from build123d import *

# Parameters (mm, degrees)
BASE_PLATE_SKETCH_W        = 120
BASE_PLATE_SKETCH_H        = 50
BASE_PLATE_120X50X10_DEPTH = 10
CLAMP_BOSS_DEPTH           = 22
BORE_SKETCH_R              = 10
BORE_20_DEPTH              = 22
COUNTERBORE_SKETCH_R       = 6
COUNTERBORES_2X_12_DEPTH   = 5
BOLT_HOLE_SKETCH_R         = 3
BOLT_HOLES_2X_6_DEPTH      = 25
MOUNTING_HOLE_SKETCH_R     = 5
MOUNTING_HOLES_4X_10_DEPTH = 25
CORNER_CHAMFERS_5MM_SIZE   = 5


with BuildPart() as part:
    # Base Plate Sketch → Base Plate 120x50x10 (new body)
    with BuildSketch(Plane.XY):
        Rectangle(BASE_PLATE_SKETCH_W, BASE_PLATE_SKETCH_H)
    extrude(amount=BASE_PLATE_120X50X10_DEPTH)

    # Clamp Boss Sketch → Clamp Boss (add)
    with BuildSketch(Plane.XY.offset(10)):
        Polygon((20, 8.3), (35, 8.3), (35, -8.3), (20, -8.3), (8.3, -20), (-8.3, -20), (-20, -8.3), (-35, -8.3), (-35, 8.3), (-20, 8.3), (-8.3, 20), (8.3, 20), align=None)
    extrude(amount=CLAMP_BOSS_DEPTH)

    # Bore Sketch → Bore Ø20 (cut)
    with BuildSketch(Plane.XY.offset(32)):
        Circle(BORE_SKETCH_R)
    extrude(amount=-BORE_20_DEPTH, mode=Mode.SUBTRACT)

    # Counterbore Sketch → Counterbores 2xØ12 (cut)
    with BuildSketch(Plane.XY.offset(32)):
        with Locations((-26, 0)):
            Circle(COUNTERBORE_SKETCH_R)
        with Locations((26, 0)):
            Circle(COUNTERBORE_SKETCH_R)
    extrude(amount=-COUNTERBORES_2X_12_DEPTH, mode=Mode.SUBTRACT)

    # Bolt Hole Sketch → Bolt Holes 2xØ6 (cut)
    with BuildSketch(Plane.XY.offset(27)):
        with Locations((-26, 0)):
            Circle(BOLT_HOLE_SKETCH_R)
        with Locations((26, 0)):
            Circle(BOLT_HOLE_SKETCH_R)
    extrude(amount=-BOLT_HOLES_2X_6_DEPTH, mode=Mode.SUBTRACT)

    # Mounting Hole Sketch → Mounting Holes 4xØ10 (cut)
    with BuildSketch(Plane.XY.offset(10)):
        with Locations((50, 15)):
            Circle(MOUNTING_HOLE_SKETCH_R)
        with Locations((50, -15)):
            Circle(MOUNTING_HOLE_SKETCH_R)
        with Locations((-50, 15)):
            Circle(MOUNTING_HOLE_SKETCH_R)
        with Locations((-50, -15)):
            Circle(MOUNTING_HOLE_SKETCH_R)
    extrude(amount=-MOUNTING_HOLES_4X_10_DEPTH, mode=Mode.SUBTRACT)

    # Corner Chamfers 5mm
    corner_chamfers_5mm_edges = [part.edges().sort_by_distance(p)[0] for p in [
        (60, -25, 5),
        (-60, -25, 5),
        (-60, 25, 5),
        (60, 25, 5),
    ]]
    chamfer(corner_chamfers_5mm_edges, length=CORNER_CHAMFERS_5MM_SIZE)


solid = part.part
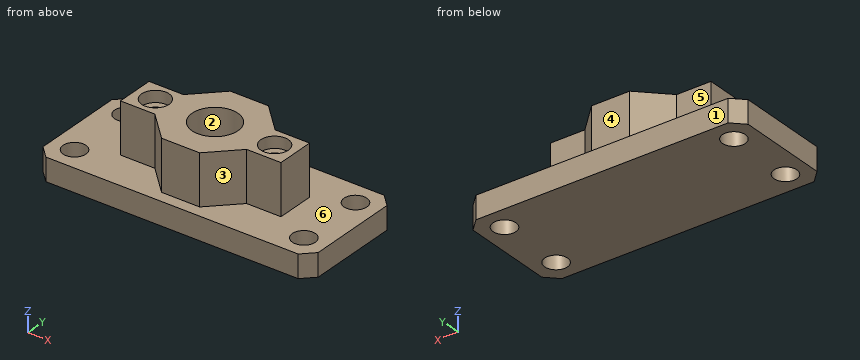
For this review, take the finished solid that the model builds, in its own axes (mm). Face numbers are marked on the shaded views. A direction names the side the tool comes from. Round coordinates to 2 decimals unless told otherwise and drop trailing zeros. Order: outer loops, then holes, each group sorted by start corner. A loop starts at its lowest first (then second) coordinate and runs counter-clockwise, first axis right, second up. Notation, with made-up numbers: (29, 60.25) -> (76, 60.25) arc R25 ccw to (76, 72.25) -> close; hole circle Ø6 at (-11.5, 63). An arc over 180 degrees is marked (long way). Write item = value, one per line. Start each with the question number.
1) The part is to be moulded in two halves that separate along X. For the marked faces 1, 2 and 3, say which applies: +X half, -X half, draft (parallel to the pull), parting line (faces both ways), or undercut.
2) Insertion check: pin 1 (4.5 mm diameter, centred on x = -28.5, z = 25.5, fed in from +Y); pin 2 (8.5 mm diameter, centred on x = 0, z = 18, fed in from +Y); pin 3 (6 mm diameter, centred on x = 4.5, y = -6, fed in from -Z); pin 4 (3 mm diameter, centred on y = -14, z = 28, fed in from -X). Each pin has a flat end and moves straight along its axis. Give the tip position at first contact, or say it passes through.
3) To check wall thickness, follow line 1 (Y direction, x = -50, z = 4.75); line 2 (X direction, y = 17.5, z = 7); line 3 (Y direction, x = 54, z = 6.5). State the ranges of each line that lie inside material, in increasing order. Write a range as from..to.
4) Take a section at A-A on x = -47. State the section outline as (y, z) points, plus the area to 3 significant figures.
5) Take a section at B-B on z = 24.5. State the section outline as (x, y) points.
6) Tool access review of the marked faces 4, 5 and 6: name each direction out of +Z, -Z, +X, -X, +Y, -Y from which nothing blocks a thin tool from reaching the whole face with its end or side.
7) Take a section at D-D on x = 26. State the section outline as (y, z) points.
8) Take a section at C-C on y = -11.5. State the section outline as (x, z) points.
Verdict:
q1.face_1 = draft
q1.face_2 = undercut
q1.face_3 = +X half
q2.pin_1 = 8.3
q2.pin_2 = 20
q2.pin_3 = 0
q2.pin_4 = -15.8
q3.line_1 = -25..-20, -10..10, 20..25
q3.line_2 = -60..-54.33, -45.67..45.67, 54.33..60
q3.line_3 = -25..-18, -12..12, 18..25
q4.outline = (-25, 0) -> (-19, 0) -> (-19, 10) -> (-25, 10) -> close; (-11, 0) -> (11, 0) -> (11, 10) -> (-11, 10) -> close; (19, 0) -> (25, 0) -> (25, 10) -> (19, 10) -> close
q4.area = 340 mm2
q5.outline = (-35, -8.3) -> (-20, -8.3) -> (-8.3, -20) -> (8.3, -20) -> (20, -8.3) -> (35, -8.3) -> (35, 8.3) -> (20, 8.3) -> (8.3, 20) -> (-8.3, 20) -> (-20, 8.3) -> (-35, 8.3) -> close; hole circle Ø6 at (-26, 0); hole circle Ø20 at (0, 0); hole circle Ø6 at (26, 0)
q6.face_4 = +Z, +X, -X, +Y
q6.face_5 = +Z, -X, +Y
q6.face_6 = +Z
q7.outline = (-25, 0) -> (25, 0) -> (25, 10) -> (8.3, 10) -> (8.3, 32) -> (6, 32) -> (6, 27) -> (3, 27) -> (3, 2) -> (-3, 2) -> (-3, 27) -> (-6, 27) -> (-6, 32) -> (-8.3, 32) -> (-8.3, 10) -> (-25, 10) -> close
q8.outline = (-60, 0) -> (-53.57, 0) -> (-53.57, 10) -> (-60, 10) -> close; (-46.43, 0) -> (46.43, 0) -> (46.43, 10) -> (16.8, 10) -> (16.8, 32) -> (-16.8, 32) -> (-16.8, 10) -> (-46.43, 10) -> close; (53.57, 0) -> (60, 0) -> (60, 10) -> (53.57, 10) -> close
